Could you check a few things on this drawing? It's one solid part, dimensions in mm from its lowest x, y, z. Give positions to 0.01 mm unless a question says otherwise; leave off trailing zeros. Write each loop counter-clockwise with the first axis right and the second up, starting at its lowest first coordinate (ties: lowest second). Pieces come first, ordered by that corner, then holes.
1. If I drill on probe 1 along X at (y, z) = (19.25, 11.5); probe 2 along Z at (x, y) = (10, 8); probe 3 along Z at (x, y) = (10, 18.75), over which ranges is the centre line in solid material (lowest first)?
2. Thinking about a two-plate mould opening in Z: for the marked faces 1, 2 and 3, which applies, pulls with the +Z half, pulls with the -Z half, needs draft (parallel to the pull), parting line crosses it, or undercut?
3. Suppose I cut it at B-B (z = 11.5). Please give me the cut outline in (x, y).
4. Suppose I cut it at C-C (y = 5). Please give me the cut outline in (x, z), and give its area (3 significant figures).
5. Suppose I cut it at D-D (z = 6.5). Please give me the cut outline in (x, y).
6. Suppose I cut it at A-A (x = 10). Please give me the cut outline in (y, z).
7. I'm going to push a flat-ended pin straight in: pin 1 (5.5 mm diameter, centred on x = 10, z = 10.5, fed in from -Y). Where does the tip first touch, or does it pass through?
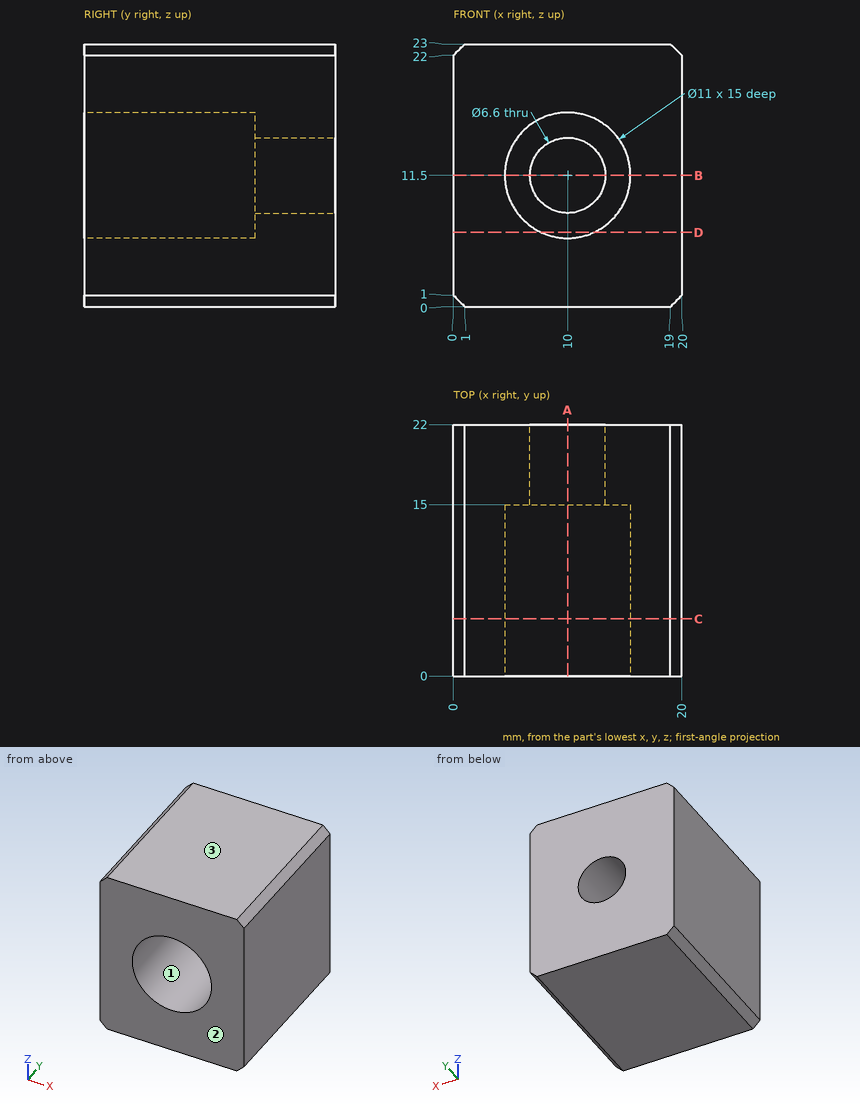
Checks:
1. probe 1: x = 0 to 6.7, 13.3 to 20
1. probe 2: z = 0 to 6, 17 to 23
1. probe 3: z = 0 to 8.2, 14.8 to 23
2. face 1: undercut
2. face 2: needs draft
2. face 3: pulls with the +Z half
3. outline: (0, 0) - (4.5, 0) - (4.5, 15) - (6.7, 15) - (6.7, 22) - (0, 22) - close; (13.3, 15) - (15.5, 15) - (15.5, 0) - (20, 0) - (20, 22) - (13.3, 22) - close
4. outline: (0, 1) - (1, 0) - (19, 0) - (20, 1) - (20, 22) - (19, 23) - (1, 23) - (0, 22) - close; hole circle Ø11 at (10, 11.5)
4. area: 363 mm2
5. outline: (0, 0) - (7.71, 0) - (7.71, 15) - (12.29, 15) - (12.29, 0) - (20, 0) - (20, 22) - (0, 22) - close
6. outline: (0, 0) - (22, 0) - (22, 8.2) - (15, 8.2) - (15, 6) - (0, 6) - close; (0, 17) - (15, 17) - (15, 14.8) - (22, 14.8) - (22, 23) - (0, 23) - close
7. pin 1: stops at y = 15
